```python
from build123d import *

# Parameters (mm, degrees)
SKETCH1_W           = 150
SKETCH1_H           = 150
BOSS_EXTRUDE1_DEPTH = 3
SKETCH2_R           = 1.44
CUT_EXTRUDE1_DEPTH  = 107.108435103
SKETCH3_R           = 1.5
CUT_EXTRUDE2_DEPTH  = 107.108435103
FILLET1_R           = 2
SKETCH4_W           = 144
SKETCH4_H           = 144
BOSS_EXTRUDE2_DEPTH = 4
CUT_EXTRUDE3_DEPTH  = 168.752794314
CUT_EXTRUDE4_DEPTH  = 168.752794314


with BuildPart() as part:
    # Sketch1 → Boss-Extrude1 (new body)
    with BuildSketch(Plane(origin=(0, 0, 0), x_dir=(1, 0, 0), z_dir=(0, 1, 0))):
        Rectangle(SKETCH1_W, SKETCH1_H)
    extrude(amount=BOSS_EXTRUDE1_DEPTH)

    # Sketch2 → Cut-Extrude1 (cut, through all)
    with BuildSketch(Plane(origin=(0, 3, 0), x_dir=(1, 0, 0), z_dir=(0, 1, 0))):
        with Locations(Location((-64.8, 65, 0), (0, 0, 270))):
            Circle(SKETCH2_R)
        with Locations(Location((-36, 65, 0), (0, 0, 270))):
            Circle(SKETCH2_R)
        with Locations(Location((-64.8, 36.2, 0), (0, 0, 270))):
            Circle(SKETCH2_R)
        with Locations(Location((-36, 36.2, 0), (0, 0, 270))):
            Circle(SKETCH2_R)
        with Locations(Location((36, 65, 0), (0, 0, 90))):
            Circle(SKETCH2_R)
        with Locations(Location((64.8, 65, 0), (0, 0, 90))):
            Circle(SKETCH2_R)
        with Locations(Location((64.8, 36.2, 0), (0, 0, 90))):
            Circle(SKETCH2_R)
        with Locations(Location((36, 36.2, 0), (0, 0, 90))):
            Circle(SKETCH2_R)
        with Locations(Location((-64.8, -36.2, 0), (0, 0, 90))):
            Circle(SKETCH2_R)
        with Locations(Location((-64.8, -65, 0), (0, 0, 90))):
            Circle(SKETCH2_R)
        with Locations(Location((-36, -65, 0), (0, 0, 90))):
            Circle(SKETCH2_R)
        with Locations(Location((-36, -36.2, 0), (0, 0, 90))):
            Circle(SKETCH2_R)
        with Locations(Location((64.8, -65, 0), (0, 0, 270))):
            Circle(SKETCH2_R)
        with Locations(Location((36, -65, 0), (0, 0, 270))):
            Circle(SKETCH2_R)
        with Locations(Location((36, -36.2, 0), (0, 0, 270))):
            Circle(SKETCH2_R)
        with Locations(Location((64.8, -36.2, 0), (0, 0, 270))):
            Circle(SKETCH2_R)
    extrude(amount=-CUT_EXTRUDE1_DEPTH, mode=Mode.SUBTRACT)

    # Sketch3 → Cut-Extrude2 (cut, through all)
    with BuildSketch(Plane(origin=(0, 3, 0), x_dir=(1, 0, 0), z_dir=(0, 1, 0))):
        with Locations(Location((-38.5, 0, 0), (0, 0, 270))):
            Circle(SKETCH3_R)
        with Locations(Location((-48.5, 10, 0), (0, 0, 270))):
            Circle(SKETCH3_R)
        with Locations(Location((-58.5, 0, 0), (0, 0, 270))):
            Circle(SKETCH3_R)
        with Locations(Location((-48.5, -10, 0), (0, 0, 270))):
            Circle(SKETCH3_R)
        with Locations(Location((-10, -48.5, 0), (0, 0, 270))):
            Circle(SKETCH3_R)
        with Locations(Location((0, -58.5, 0), (0, 0, 270))):
            Circle(SKETCH3_R)
        with Locations(Location((10, -48.5, 0), (0, 0, 270))):
            Circle(SKETCH3_R)
        with Locations(Location((0, -38.5, 0), (0, 0, 270))):
            Circle(SKETCH3_R)
        with Locations(Location((58.5, 0, 0), (0, 0, 270))):
            Circle(SKETCH3_R)
        with Locations(Location((48.5, 10, 0), (0, 0, 270))):
            Circle(SKETCH3_R)
        with Locations(Location((38.5, 0, 0), (0, 0, 270))):
            Circle(SKETCH3_R)
        with Locations(Location((0, 38.5, 0), (0, 0, 270))):
            Circle(SKETCH3_R)
        with Locations(Location((10, 48.5, 0), (0, 0, 270))):
            Circle(SKETCH3_R)
        with Locations(Location((0, 58.5, 0), (0, 0, 270))):
            Circle(SKETCH3_R)
        with Locations(Location((-10, 48.5, 0), (0, 0, 270))):
            Circle(SKETCH3_R)
        with Locations(Location((48.5, -10, 0), (0, 0, 270))):
            Circle(SKETCH3_R)
    extrude(amount=-CUT_EXTRUDE2_DEPTH, mode=Mode.SUBTRACT)

    # Fillet1
    fillet1_edges = [part.edges().sort_by_distance(p)[0] for p in [
        (75, 1.5, 75),
        (-75, 1.5, 75),
        (-75, 1.5, -75),
        (75, 1.5, -75),
    ]]
    fillet(fillet1_edges, radius=FILLET1_R)

    # Sketch4 → Boss-Extrude2 (add)
    with BuildSketch(Plane.XZ):
        with BuildLine():
            Line((73, -75), (-73, -75))
            ThreePointArc((-73, -75), (-74.414213562, -74.414213562), (-75, -73))
            Line((-75, -73), (-75, 73))
            ThreePointArc((-75, 73), (-74.414213562, 74.414213562), (-73, 75))
            Line((-73, 75), (73, 75))
            ThreePointArc((73, 75), (74.414213562, 74.414213562), (75, 73))
            Line((75, 73), (75, -73))
            ThreePointArc((75, -73), (74.414213562, -74.414213562), (73, -75))
        make_face()
        Rectangle(SKETCH4_W, SKETCH4_H, mode=Mode.SUBTRACT)
    extrude(amount=BOSS_EXTRUDE2_DEPTH)

    # Sketch5 → Cut-Extrude3 (cut, through all)
    with BuildSketch(Plane.XY.offset(75)):
        Polygon((-55, -4), (-51, 0), (51, 0), (55, -4), align=None)
    extrude(amount=-CUT_EXTRUDE3_DEPTH, mode=Mode.SUBTRACT)

    # Sketch6 → Cut-Extrude4 (cut, through all)
    with BuildSketch(Plane.ZY.offset(75)):
        Polygon((-55, -4), (-51, 0), (51, 0), (55, -4), align=None)
    extrude(amount=-CUT_EXTRUDE4_DEPTH, mode=Mode.SUBTRACT)


solid = part.part
```
Model file for the job. Use its own axes, mm. A direction names the side the tool comes from. Coordinates: 2 decimals unless noted, no trailing zeros. Order: outer loops, then holes, each group sorted by start corner. A loop starts at its lowest first (then second) coordinate and runs counter-clockwise, first axis right, second up. Notation, with made-up numbers: M 28,-8 L 38,-8 A11 cw 38,10 Z; hole C 79.5,-28 d10. An arc over 180 degrees is marked long. Answer as CSV lines item,"result".
(1) Band-saw the part on A-A, the plane y = -1.75. List the corners of the cut face in (x, z), then the cut area to 3 significant figures.
Geometry says:
outline,"M -75,-73 A2 ccw -73,-75 L -52.75,-75 L -52.75,-72 L -72,-72 L -72,-52.75 L -75,-52.75 Z; M -75,52.75 L -72,52.75 L -72,72 L -52.75,72 L -52.75,75 L -73,75 A2 ccw -75,73 Z; M 52.75,-75 L 73,-75 A2 ccw 75,-73 L 75,-52.75 L 72,-52.75 L 72,-72 L 52.75,-72 Z; M 52.75,72 L 72,72 L 72,52.75 L 75,52.75 L 75,73 A2 ccw 73,75 L 52.75,75 Z"
area,"495 mm2"
(2) Pull direction X, two halves, no side cores. Call faces 1 (the flat face through (75, 1, 1)), 2 (the flat face through (-53, -2, 74)), 3 (the flat face through (-1, 3, -1)): +X half, -X half, draft (parallel to the pull), parting line (faces both ways), or undercut.
Geometry says:
face 1,"+X half"
face 2,"undercut"
face 3,"draft"
(3) Band-saw the part on B-B, the plane z = -30. List the corners of the cut face in (x, y).
Geometry says:
outline,"M -75,0 L 75,0 L 75,3 L -75,3 Z"
(4) Wall check: line 1 along X through (y, z) = (2.1, -65); line 2 along Z through (x, y) = (-64.8, 2); line 3 along X through (y, z) = (0.6, -48.5). Give the ranges that are in metal, low to high.
Geometry says:
line 1,"x = -75 to -66.24, -63.36 to -37.44, -34.56 to 34.56, 37.44 to 63.36, 66.24 to 75"
line 2,"z = -75 to -66.44, -63.56 to -37.64, -34.76 to 34.76, 37.64 to 63.56, 66.44 to 75"
line 3,"x = -75 to -11.5, -8.5 to 8.5, 11.5 to 75"
(5) Flat gauge pin, fed straight in: pin 1 (4 mm diameter, centred on x = 10, z = 48.5, fed in from -Y). Where does the tip first touch, or does it go through?
Geometry says:
pin 1,"stops at y = 0"
(6) 3-axis set-ups, long thin cutter, end or side, ignore diameter. For faces 4 (the flat face through (61, -2, -72)), 5 (the flat face through (-1, 1, 75)), 6 (the flat face through (53, -2, -73)), 7 (the flat face through (-74, -2, 53)): which of +Z, -Z, +X, -X, +Y, -Y reach the whole face in a straight line?
Geometry says:
face 4,"-Y"
face 5,"+Z, +X, -X, +Y, -Y"
face 6,"+Z, -Z, -Y"
face 7,"+X, -X, -Y"
